Geometry check sheet. Reference: the model listing, model coordinates, mm. Face numbers are marked on the shaded views. A direction names the side the tool comes from. Coordinates: 2 decimals unless noted, no trailing zeros. Loops run counter-clockwise (first coordinate to the right, second up) from the corner with the lowest first, then second, coordinate; pieces in that order, holes last.
from build123d import *

# Parameters (mm, degrees)
SKETCH1_W                                           = 10.3
SKETCH1_H                                           = 7
BOSS_EXTRUDE1_DEPTH                                 = 29
FILLET1_RADIUS                                      = 5.15
FILLET1_LENGTH                                      = 7
FILLET2_RADIUS                                      = 5.15
FILLET2_LENGTH                                      = 7
CHAMFER1_SIZE                                       = 0.5
HOLE_SPEC_PER_SOCKET_HEAD_CAP_SCREW_TYP_D           = 3.4
HOLE_SPEC_PER_SOCKET_HEAD_CAP_SCREW_TYP_CBORE_D     = 6
HOLE_SPEC_PER_SOCKET_HEAD_CAP_SCREW_TYP_CBORE_DEPTH = 3.4


with BuildPart() as part:
    # Sketch1 → Boss-Extrude1 (new body)
    with BuildSketch(Plane.XY):
        Rectangle(SKETCH1_W, SKETCH1_H)
    extrude(amount=BOSS_EXTRUDE1_DEPTH)

    # Fillet1: full round fillet: the end face becomes a half cylinder, R = half its width
    fillet1_face = Plane((0, 0, 0), x_dir=(0, 1, 0), z_dir=(0, 0, -1))  # on the end face: x along it, z out of the body
    fillet1_slab = fillet1_face.offset(-FILLET1_RADIUS / 2) * Box(FILLET1_LENGTH, 2 * FILLET1_RADIUS, FILLET1_RADIUS, mode=Mode.PRIVATE)  # the body's end, R deep
    fillet1_round = Plane((0, 0, 5.15), x_dir=(0, 0, -1), z_dir=(0, 1, 0)) * Cylinder(FILLET1_RADIUS, FILLET1_LENGTH, mode=Mode.PRIVATE)  # its axis R under the face
    add(fillet1_slab - fillet1_round, mode=Mode.SUBTRACT)

    # Fillet2: full round fillet: the end face becomes a half cylinder, R = half its width
    fillet2_face = Plane((0, 0, 29), x_dir=(0, -1, 0), z_dir=(0, 0, 1))  # on the end face: x along it, z out of the body
    fillet2_slab = fillet2_face.offset(-FILLET2_RADIUS / 2) * Box(FILLET2_LENGTH, 2 * FILLET2_RADIUS, FILLET2_RADIUS, mode=Mode.PRIVATE)  # the body's end, R deep
    fillet2_round = Plane((0, 0, 23.85), x_dir=(0, 0, 1), z_dir=(0, -1, 0)) * Cylinder(FILLET2_RADIUS, FILLET2_LENGTH, mode=Mode.PRIVATE)  # its axis R under the face
    add(fillet2_slab - fillet2_round, mode=Mode.SUBTRACT)

    # Chamfer1
    chamfer1_edges = [part.edges().sort_by_distance(p)[0] for p in [
        (0, -3.5, 0),
        (0, 3.5, 0),
        (5.15, -3.5, 14.5),
        (5.15, 3.5, 14.5),
        (-5.15, 3.5, 14.5),
        (-5.15, -3.5, 14.5),
        (0, 3.5, 29),
        (0, -3.5, 29),
    ]]
    chamfer(chamfer1_edges, length=CHAMFER1_SIZE)

    # Hole Spec (per socket head cap screw type) 1 (through all)
    with Locations(Plane(origin=(0, 3.5, 0), x_dir=(1, 0, 0), z_dir=(0, 1, 0))):
        with Locations((0, -24.5), (0, -4.5)):
            CounterBoreHole(HOLE_SPEC_PER_SOCKET_HEAD_CAP_SCREW_TYP_D / 2, HOLE_SPEC_PER_SOCKET_HEAD_CAP_SCREW_TYP_CBORE_D / 2, HOLE_SPEC_PER_SOCKET_HEAD_CAP_SCREW_TYP_CBORE_DEPTH)


solid = part.part
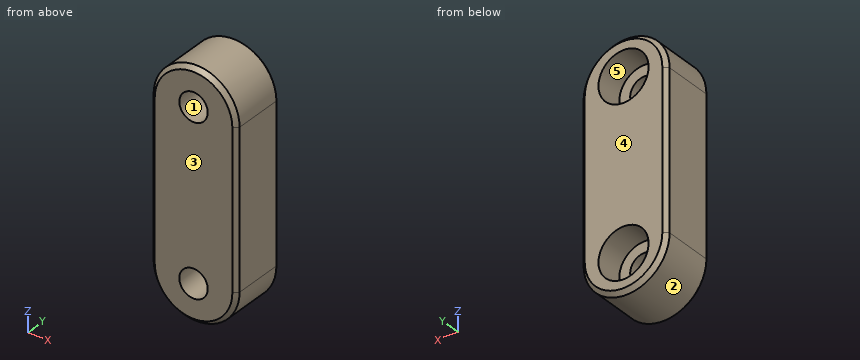
1) Depth check by flat-ended pin: pin 1 (5 mm diameter, centred on x = 0, z = 24.5, fed in from -Y); pin 2 (3 mm diameter, centred on x = -2, y = -0.5, fed in from -Z); pin 3 (1.8 mm diameter, centred on x = 0, z = 3, fed in from +Y). Enter the tip coordinate at first touch or a pass-through.
Data:
pin 1: stops at y = -3.5
pin 2: stops at z = 0.02
pin 3: stops at y = 0.1
2) Mould release check, pull along Z, two halves, no side actions. Record for the marked faces 1, 2 and 3: +Z half, -Z half, draft (parallel to the pull), parting line (faces both ways), or undercut.
Data:
face 1: undercut
face 2: -Z half
face 3: draft
3) Section check A-A on x = 0. Record the cut outline in (y, z).
Data:
outline: (-3.5, 0.5) - (-3, 0) - (3, 0) - (3.5, 0.5) - (3.5, 1.5) - (0.1, 1.5) - (0.1, 2.8) - (-3.5, 2.8) - close; (-3.5, 6.2) - (0.1, 6.2) - (0.1, 7.5) - (3.5, 7.5) - (3.5, 21.5) - (0.1, 21.5) - (0.1, 22.8) - (-3.5, 22.8) - close; (-3.5, 26.2) - (0.1, 26.2) - (0.1, 27.5) - (3.5, 27.5) - (3.5, 28.5) - (3, 29) - (-3, 29) - (-3.5, 28.5) - close
4) Section check C-C on z = 7. Record the cut outline in (x, y).
Data:
outline: (-5.15, -3) - (-4.65, -3.5) - (4.65, -3.5) - (5.15, -3) - (5.15, 3) - (4.65, 3.5) - (1.66, 3.5) - (1.66, 0.1) - (-1.66, 0.1) - (-1.66, 3.5) - (-4.65, 3.5) - (-5.15, 3) - close
5) Section check D-D on y = 2.5. Record the cut outline in (x, z).
Data:
outline: (-5.15, 5.15) arc R5.15 ccw to (5.15, 5.15) - (5.15, 23.85) arc R5.15 ccw to (-5.15, 23.85) - close; hole circle Ø6 at (0, 4.5); hole circle Ø6 at (0, 24.5)
6) Section check B-B on y = -1. Record the cut outline in (x, z).
Data:
outline: (-5.15, 5.15) arc R5.15 ccw to (5.15, 5.15) - (5.15, 23.85) arc R5.15 ccw to (-5.15, 23.85) - close; hole circle Ø3.4 at (0, 4.5); hole circle Ø3.4 at (0, 24.5)
7) Material ranges on probe 1 along Z at (x, y) = (0, -2.1); probe 2 along Z at (x, y) = (0, 2.7); probe 3 along Y at (x, z) = (0, 7.25), recorded low to high.
Data:
probe 1: z = 0 to 2.8, 6.2 to 22.8, 26.2 to 29
probe 2: z = 0 to 1.5, 7.5 to 21.5, 27.5 to 29
probe 3: y = -3.5 to 0.1
8) Access from +Z, -Z, +X, -X, +Y, -Y to the whole of each face (thin tool, end or side, straight path). Record for the marked faces 4 and 5.
Data:
face 4: +Z, -Z, +X, -X, +Y
face 5: +Y
